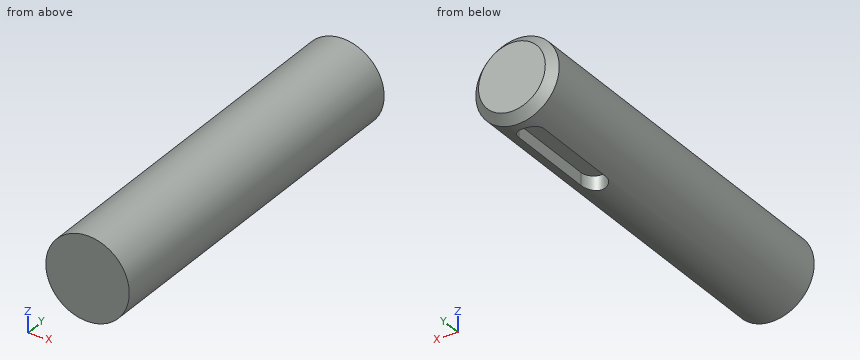
```python
from build123d import *

# Parameters (mm, degrees)
SKETCH_1_R           = 10
BOSS_EXTRUDE_1_DEPTH = 92.5
CUT_EXTRUDE_1_DEPTH  = 95.490740287
CHAMFER_1_SIZE       = 2


with BuildPart() as part:
    # Sketch 1 → Boss-Extrude 1 (new body)
    with BuildSketch(Plane(origin=(0, 0, 0), x_dir=(1, 0, 0), z_dir=(0, 1, 0))):
        with Locations(Location((0, 0, 0), (0, 0, 270))):
            Circle(SKETCH_1_R)
    extrude(amount=BOSS_EXTRUDE_1_DEPTH)

    # Sketch 2 → Cut-Extrude 1 (cut, through all)
    with BuildSketch(Plane.XY.offset(-6.5)):
        with BuildLine():
            Line((-3, 63.5), (-3, 85.5))
            ThreePointArc((-3, 85.5), (0, 88.5), (3, 85.5))
            Line((3, 85.5), (3, 63.5))
            ThreePointArc((3, 63.5), (0, 60.5), (-3, 63.5))
        make_face()
    extrude(amount=-CUT_EXTRUDE_1_DEPTH, mode=Mode.SUBTRACT)

    # Chamfer 1
    chamfer_1_edges = [part.edges().sort_by_distance(p)[0] for p in [
        (0, 92.5, -10),
    ]]
    chamfer(chamfer_1_edges, length=CHAMFER_1_SIZE)


solid = part.part
```
Read the model definition and answer for the solid it produces. Units are mm, in the model's axes. Give positions to 0.01 mm unless a question says otherwise; leave off trailing zeros. Write each loop counter-clockwise with the first axis right and the second up, starting at its lowest first coordinate (ties: lowest second). Pieces come first, ordered by that corner, then holes. Notation, with made-up numbers: M 34,-26.75 L 60,-26.75 A23 ccw 60,-1.75 Z; hole C 55,64.25 d9. An arc over 180 degrees is marked long. Put each result on its own line as item: value. Start each with the question number.
1. Each of these flat-tipped pins is pushed along its axis until it touches: pin 1 Ø2.5 at (y, z) = (69.5, -8.5) entering from +X; pin 2 Ø6 at (x, y) = (7.5, 10.5) entering from -Z; pin 3 Ø8 at (y, z) = (35, 4.5) entering from +X. Where does it stop, or does it pass through?
2. The part is cut by section A-A, the plane x = 0. Give the vertices of the cut face in (y, z), and give its area (3 significant figures).
3. The part is cut by section C-C, the plane y = 6. Give the vertices of the cut face in (x, z), and give its area (3 significant figures).
4. Consider line 1 along Z through (x, y) = (-0.25, 37); line 2 along Z through (x, y) = (-2.5, 80); line 3 along X through (y, z) = (13, -8). Determine where each line is inside the solid, lowest interval first.
5. The part is cut by section B-B, the plane y = 77.5. Give the vertices of the cut face in (x, z), and give its area (3 significant figures).
Final values:
1. pin 1: stops at x = 6.89
1. pin 2: stops at z = -8.93
1. pin 3: stops at x = 9.99
2. outline: M 0,-10 L 60.5,-10 L 60.5,-6.5 L 88.5,-6.5 L 88.5,-10 L 90.5,-10 L 92.5,-8 L 92.5,8 L 90.5,10 L 0,10 Z
2. area: 1,750 mm²
3. outline: C 0,0 d20
3. area: 314 mm²
4. line 1: z = -10 to 10
4. line 2: z = -6.5 to 9.68
4. line 3: x = -6 to 6
5. outline: M -3,-9.54 L -3,-6.5 L 3,-6.5 L 3,-9.54 A10 ccw long Z
5. area: 294 mm²
